Read the model definition and answer for the solid it produces. Units are mm, in the model's axes. Face numbers are marked on the shaded views. A direction names the side the tool comes from. Coordinates: 2 decimals unless noted, no trailing zeros. Loops run counter-clockwise (first coordinate to the right, second up) from the corner with the lowest first, then second, coordinate; pieces in that order, holes last. Notation, with made-up numbers: (2, 43.25) -> (43, 43.25) arc R17 ccw to (43, 76.25) -> close; hole circle Ø5 at (62.5, -1.75). An arc over 180 degrees is marked (long way). Answer in a Markdown table with one row per item.
```python
from build123d import *

# Parameters (mm, degrees)
EXTRUDE_1_DEPTH     = 10
SKETCH_2_R          = 20
EXTRUDE_2_DEPTH     = 10
SKETCH_3_R          = 19.9
EXTRUDE_3_DEPTH     = 61
SKETCH_5_R          = 12.5
CUT_EXTRUDE_1_DEPTH = 90.997866916
SKETCH_6_R          = 3.3
CUT_EXTRUDE_2_DEPTH = 90.997866916
CHAMFER_1_SIZE      = 0.5


with BuildPart() as part:
    # 草图1 → 拉伸1 (new body)
    with BuildSketch(Plane(origin=(0, 0, 0), x_dir=(1, 0, 0), z_dir=(0, 1, 0))):
        with BuildLine():
            Line((24, -19.595362506), (24, 19.647471235))
            ThreePointArc((24, 19.647471235), (0, 31.026054364), (-24, 19.647471235))
            Line((-24, 19.647471235), (-24, -19.595362506))
            ThreePointArc((-24, -19.595362506), (0, -30.973945636), (24, -19.595362506))
        make_face()
    extrude(amount=EXTRUDE_1_DEPTH)

    # 草图2 → 拉伸2 (add)
    with BuildSketch(Plane(origin=(0, 10, 0), x_dir=(-1, 0, 0), z_dir=(0, 1, 0))):
        with Locations(Location((0, 0, 0), (0, 0, 90))):
            Circle(SKETCH_2_R)
    extrude(amount=EXTRUDE_2_DEPTH)

    # 草图3 → 拉伸3 (add)
    with BuildSketch(Plane(origin=(0, 20, 0), x_dir=(-1, 0, 0), z_dir=(0, 1, 0))):
        with Locations(Location((0, 0, 0), (0, 0, 270))):
            Circle(SKETCH_3_R)
    extrude(amount=EXTRUDE_3_DEPTH)

    # 草图5 → 切除-拉伸1 (cut, through all)
    with BuildSketch(Plane(origin=(0, 81, 0), x_dir=(-1, 0, 0), z_dir=(0, 1, 0))):
        with Locations(Location((0, 0, 0), (0, 0, 90))):
            Circle(SKETCH_5_R)
    extrude(amount=-CUT_EXTRUDE_1_DEPTH, mode=Mode.SUBTRACT)

    # 草图6 → 切除-拉伸2 (cut, through all)
    with BuildSketch(Plane.XZ):
        with Locations(Location((18.03122292, -18.03122292, 0), (0, 0, 270))):
            Circle(SKETCH_6_R)
        with Locations(Location((0, -25.5, 0), (0, 0, 270))):
            Circle(SKETCH_6_R)
        with Locations(Location((-18.03122292, -18.03122292, 0), (0, 0, 270))):
            Circle(SKETCH_6_R)
        with Locations(Location((-18.03122292, 18.03122292, 0), (0, 0, 270))):
            Circle(SKETCH_6_R)
        with Locations(Location((0, 25.5, 0), (0, 0, 270))):
            Circle(SKETCH_6_R)
        with Locations(Location((18.03122292, 18.03122292, 0), (0, 0, 270))):
            Circle(SKETCH_6_R)
    extrude(amount=-CUT_EXTRUDE_2_DEPTH, mode=Mode.SUBTRACT)

    # 倒角1
    chamfer_1_edges = [part.edges().sort_by_distance(p)[0] for p in [
        (0, 81, 19.9),
    ]]
    chamfer(chamfer_1_edges, length=CHAMFER_1_SIZE)


solid = part.part
```
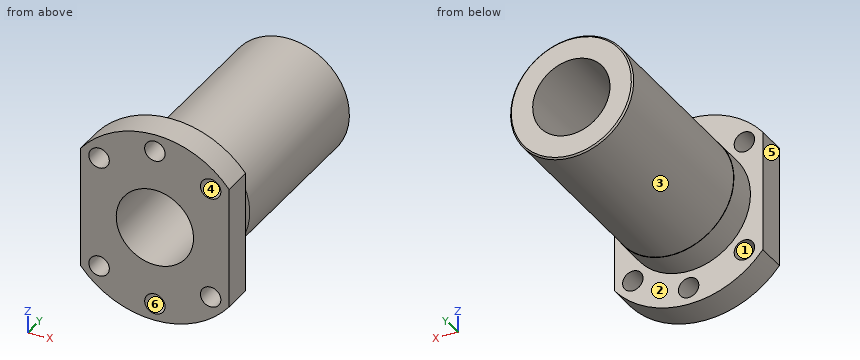
1. A cutting plane is placed at B-B on z = 0. Give the vertices of the cut face in (x, y).
A:
| item | result |
|---|---|
| outline | (-24, 0) -> (-12.5, 0) -> (-12.5, 81) -> (-19.4, 81) -> (-19.9, 80.5) -> (-19.9, 20) -> (-20, 20) -> (-20, 10) -> (-24, 10) -> close; (12.5, 0) -> (24, 0) -> (24, 10) -> (20, 10) -> (20, 20) -> (19.9, 20) -> (19.9, 80.5) -> (19.4, 81) -> (12.5, 81) -> close |
2. A cutting plane is placed at A-A on x = 0. Give the vertices of the cut face in (y, z), and give its area (3 significant figures).
A:
| item | result |
|---|---|
| outline | (0, -31.03) -> (10, -31.03) -> (10, -28.8) -> (0, -28.8) -> close; (0, -22.2) -> (10, -22.2) -> (10, -20) -> (20, -20) -> (20, -19.9) -> (80.5, -19.9) -> (81, -19.4) -> (81, -12.5) -> (0, -12.5) -> close; (0, 12.5) -> (81, 12.5) -> (81, 19.4) -> (80.5, 19.9) -> (20, 19.9) -> (20, 20) -> (10, 20) -> (10, 22.2) -> (0, 22.2) -> close; (0, 28.8) -> (10, 28.8) -> (10, 30.97) -> (0, 30.97) -> close |
| area | 1,290 mm2 |
3. The mould has two halves that part along X. Classify the marked faces 3, 4, 5 and 6: pulls with the +X half, pulls with the -X half, needs draft (parallel to the pull), parting line crosses it, or undercut.
A:
| item | result |
|---|---|
| face 3 | parting line crosses it |
| face 4 | undercut |
| face 5 | pulls with the -X half |
| face 6 | undercut |
4. A cutting plane is placed at D-D on z = 25.5. Give the vertices of the cut face in (x, y).
A:
| item | result |
|---|---|
| outline | (-17.59, 0) -> (-3.3, 0) -> (-3.3, 10) -> (-17.59, 10) -> close; (3.3, 0) -> (17.59, 0) -> (17.59, 10) -> (3.3, 10) -> close |
5. Given pin 1 Ø6 at (x, z) = (0, -25.5) entering from +Y; pin 2 Ø5 at (y, z) = (60, 18.5) entering from -X; pin 3 Ø10.5 at (x, z) = (18.03, -18.03) entering from +Y; pin 4 Ø6 at (x, y) = (-3.5, 13.5) entering from +Z, each flat-ended and moving along its own axis, determine where each tip first touches the part or whether it passes through.
A:
| item | result |
|---|---|
| pin 1 | passes through |
| pin 2 | stops at x = -11.83 |
| pin 3 | stops at y = 10 |
| pin 4 | stops at z = 19.99 |
6. A tool of negligible diameter and unlimited length cuts with its end or side. For the marked faces 1 and 2, from which of +Z, -Z, +X, -X, +Y, -Y can it reach the whole face along a straight path? Write none if from no direction.
A:
| item | result |
|---|---|
| face 1 | +Y, -Y |
| face 2 | +Y |
7. Find the intervals of material crossed by probe 1 along Y at (x, z) = (13.5, 16); probe 2 along Z at (x, y) = (-7, 16.5) (3 decimals); probe 3 along X at (y, z) = (64, 0), in increasing order.
A:
| item | result |
|---|---|
| probe 1 | y = 0 to 10 |
| probe 2 | z = -18.735 to -10.356, 10.356 to 18.735 |
| probe 3 | x = -19.9 to -12.5, 12.5 to 19.9 |
8. A cutting plane is placed at C-C on y = 39. Give the vertices of the cut face in (x, z).
A:
| item | result |
|---|---|
| outline | circle Ø39.8 at (0, 0); hole circle Ø25 at (0, 0) |
